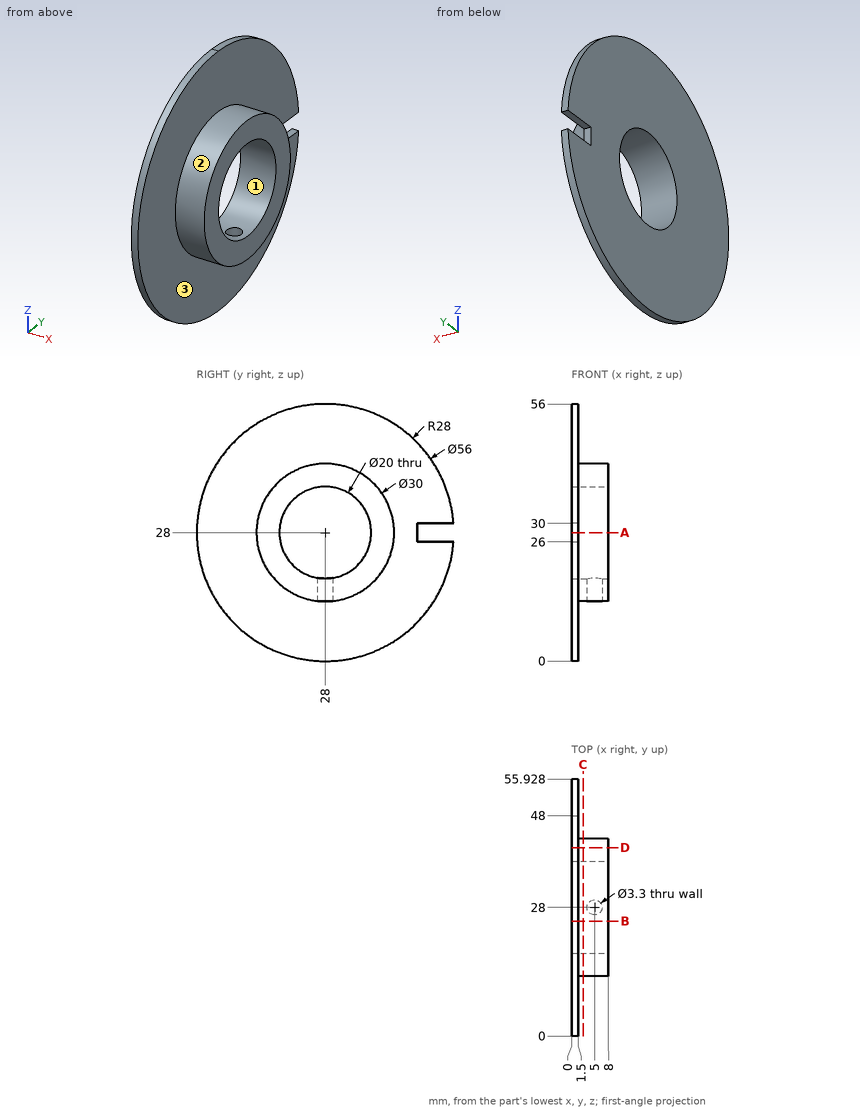
Study the drawing (mm; zero at the part's minimum x, y, z) and answer. Give positions to 0.01 mm unless a question says otherwise; leave off trailing zeros. Order: outer loops, then holes, each group sorted by start corner. A loop starts at its lowest first (then second) coordinate and runs counter-clockwise, first axis right, second up.
1. Section B-B, the plane y = 25 is taken. Determine the outline of the cut face in (x, z), and give its area (3 significant figures).
Result sheet:
outline: (0, 0.16) - (1.5, 0.16) - (1.5, 13.3) - (8, 13.3) - (8, 18.46) - (0, 18.46) - close; (0, 37.54) - (8, 37.54) - (8, 42.7) - (1.5, 42.7) - (1.5, 55.84) - (0, 55.84) - close
area: 122 mm2
2. Section D-D, the plane y = 41 is taken. Determine the outline of the cut face in (x, z), and give its area (3 significant figures).
Result sheet:
outline: (0, 3.2) - (1.5, 3.2) - (1.5, 20.52) - (8, 20.52) - (8, 35.48) - (1.5, 35.48) - (1.5, 52.8) - (0, 52.8) - close
area: 172 mm2
3. Section C-C, the plane x = 2.5 is taken. Determine the outline of the cut face in (y, z), and give its area (3 significant figures).
Result sheet:
outline: circle Ø30 at (28, 28); hole circle Ø20 at (28, 28)
area: 393 mm2
4. Each of these flat-tipped pins is pushed along its axis until it touches: P1, Ø0.8, axis at x = 1, y = 52, coming from the -Z side; P2, Ø4, axis at x = 4.5, z = 15.5, coming from the -Y side; P3, Ø1.5, axis at x = 2.5, y = 17.5, coming from the +Z side. Where does it stop, or does it pass through?
Result sheet:
P1: stops at z = 12.93
P2: stops at y = 17.29
P3: stops at z = 39.4
5. Straight lines are drawn through the part: L1, parallel to Y at x = 4.25, z = 28; L2, parallel to X at y = 53.5, z = 36.5. For each, find the intervals that lie inside material, in ascending order.
Result sheet:
L1: y = 13 to 18, 38 to 43
L2: x = 0 to 1.5
6. The mould has two halves that part along Y. Classify the marked faces 1, 2 and 3: released by +Y, released by -Y, zero draft, split by the parting line, or undercut.
Result sheet:
face 1: undercut
face 2: split by the parting line
face 3: zero draft
7. Section A-A, the plane z = 28 is taken. Determine the outline of the cut face in (x, y), and give its area (3 significant figures).
Result sheet:
outline: (0, 0) - (1.5, 0) - (1.5, 13) - (8, 13) - (8, 18) - (0, 18) - close; (0, 38) - (8, 38) - (8, 43) - (1.5, 43) - (1.5, 48) - (0, 48) - close
area: 107 mm2
